```python
from build123d import *

# Parameters (mm, degrees)
SKETCH1_R           = 25
BOSS_EXTRUDE1_DEPTH = 20


with BuildPart() as part:
    # Sketch1 → Boss-Extrude1 (new body)
    with BuildSketch(Plane.XY):
        with BuildLine():
            Line((122.728358581, 80), (308.159136141, 49.329793203))
            ThreePointArc((308.159136141, 49.329793203), (350, 0), (308.159136141, -49.329793203))
            Line((308.159136141, -49.329793203), (122.728358581, -80))
            ThreePointArc((122.728358581, -80), (-146.5, 0), (122.728358581, 80))
        make_face()
        with Locations((300, 0)):
            Circle(SKETCH1_R, mode=Mode.SUBTRACT)
    extrude(amount=BOSS_EXTRUDE1_DEPTH)


solid = part.part
```
Can you work these out from the model? Positions are in its coordinate system, mm. Give positions to 0.01 mm unless a question says otherwise; leave off trailing zeros. Order: outer loops, then holes, each group sorted by start corner. A loop starts at its lowest first (then second) coordinate and runs counter-clockwise, first axis right, second up. Notation, with made-up numbers: (-34.75, 76.5) - (14.25, 76.5) arc R10 cw to (14.25, 80.5) - close; hole circle Ø2 at (6, -15.75). An arc over 180 degrees is marked (long way). Use a Markdown table: item, result. Add a question column.
Q1. If we section it at B-B on z = 10.5: Write out the boundary of the cut face in (x, y).
Q2. If we section it at D-D on y = 65: Write out the boundary of the cut face in (x, z), plus the area to 3 significant figures.
Q3. If we section it at C-C on x = 300: Write out the boundary of the cut face in (y, z), plus the area to 3 significant figures.
Q4. I'm going to push flat-ended pins straight in: pin 1 (4 mm diameter, centred on y = -104.5, z = 16, fed in from -X); pin 2 (6 mm diameter, centred on x = 298.5, z = 8.5, fed in from -Y); pin 3 (10 mm diameter, centred on y = -45.5, z = 3.5, fed in from +X). Where does each tip first touch, or does it pass through?
Q5. Please list where these lines run through material, in increasing order: line 1 along X through (y, z) = (2, 11.25); line 2 along Y through (x, z) = (300, 4.5); line 3 along Y through (x, z) = (-10, 5).
Q6. If we mould it in two halves opening along Y, with no side actions, what happens to faces 1 (the cylindrical face through (323.846, 7.509, 9.86)), 2 (the flat face through (50, 2, 0)), 3 (the cylindrical face through (349.99, 0.98, 9.86))? For each: released by +Y, released by -Y, zero draft, split by the parting line, or undercut.
Q7. If we section it at A-A on y = 0: Write out the boundary of the cut face in (x, z), plus the area to 3 significant figures.
Answers follow:
| question | item | result |
|---|---|---|
| 1 | outline | (122.73, -80) - (308.16, -49.33) arc R50 ccw to (308.16, 49.33) - (122.73, 80) arc R146.5 ccw (long way) to start; hole circle Ø50 at (300, 0) |
| 2 | outline | (-131.29, 0) - (213.42, 0) - (213.42, 20) - (-131.29, 20) - close |
| 2 | area | 6,890 mm^2 |
| 3 | outline | (-50.68, 0) - (-25, 0) - (-25, 20) - (-50.68, 20) - close; (25, 0) - (50.68, 0) - (50.68, 20) - (25, 20) - close |
| 3 | area | 1,030 mm^2 |
| 4 | pin 1 | stops at x = -104.67 |
| 4 | pin 2 | stops at y = -51.42 |
| 4 | pin 3 | stops at x = 329.32 |
| 5 | line 1 | x = -146.49 to 275.08, 324.92 to 349.96 |
| 5 | line 2 | y = -50.68 to -25, 25 to 50.68 |
| 5 | line 3 | y = -146.16 to 146.16 |
| 6 | face 1 | undercut |
| 6 | face 2 | zero draft |
| 6 | face 3 | split by the parting line |
| 7 | outline | (-146.5, 0) - (275, 0) - (275, 20) - (-146.5, 20) - close; (325, 0) - (350, 0) - (350, 20) - (325, 20) - close |
| 7 | area | 8,930 mm^2 |
